from build123d import *

# Parameters (mm, degrees)
SKETCH2_R           = 31
BOSS_EXTRUDE1_DEPTH = 3
SKETCH3_R           = 22.5
BOSS_EXTRUDE2_DEPTH = 12
SKETCH4_R           = 17.5
CUT_EXTRUDE1_DEPTH  = 9
SKETCH6_R           = 2.75
CUT_EXTRUDE2_DEPTH  = 12


with BuildPart() as part:
    # Sketch2 → Boss-Extrude1 (new body)
    with BuildSketch(Plane.XY.offset(-694.189912682)):
        with Locations((-50, 0)):
            Circle(SKETCH2_R)
    extrude(amount=BOSS_EXTRUDE1_DEPTH)

    # Sketch3 → Boss-Extrude2 (add)
    with BuildSketch(Plane(origin=(0, 0, -694.189912682), x_dir=(-1, 0, 0), z_dir=(0, 0, -1))):
        with Locations((50, 0)):
            Circle(SKETCH3_R)
    extrude(amount=BOSS_EXTRUDE2_DEPTH)

    # Sketch4 → Cut-Extrude1 (cut)
    with BuildSketch(Plane(origin=(0, 0, -706.189912682), x_dir=(-1, 0, 0), z_dir=(0, 0, -1))):
        with Locations((50, 0)):
            Circle(SKETCH4_R)
    extrude(amount=-CUT_EXTRUDE1_DEPTH, mode=Mode.SUBTRACT)

    # Sketch6 → Cut-Extrude2 (cut)
    with BuildSketch(Plane.XY.offset(-691.189912682)):
        with Locations((-50, 26)):
            Circle(SKETCH6_R)
        with Locations((-24, 0)):
            Circle(SKETCH6_R)
        with Locations((-50, -26)):
            Circle(SKETCH6_R)
        with Locations((-76, 0)):
            Circle(SKETCH6_R)
    extrude(amount=-CUT_EXTRUDE2_DEPTH, mode=Mode.SUBTRACT)


solid = part.part
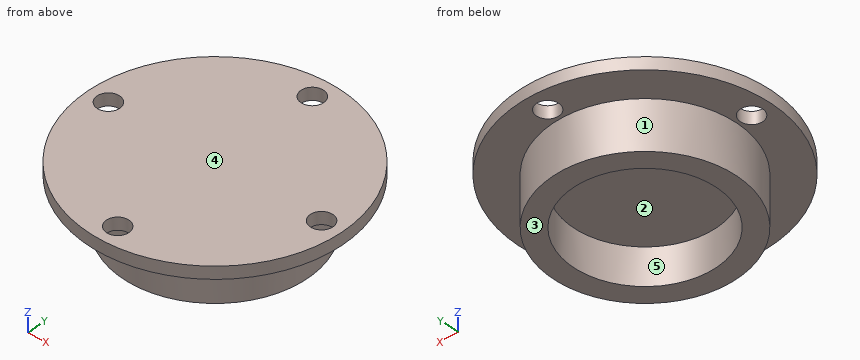
Work out the finished part from the listing and answer in its coordinate system (mm). Face numbers are marked on the shaded views. A direction names the side the tool comes from. Round coordinates to 2 decimals unless told otherwise and drop trailing zeros. Loops run counter-clockwise (first coordinate to the right, second up) from the corner with the lowest first, then second, coordinate; pieces in that order, holes last. Notation, with made-up numbers: (72.25, 72.25) - (94.25, 72.25) arc R18 cw to (94.25, 80.25) - close; hole circle Ø3 at (-24.5, 64). An arc over 180 degrees is marked (long way). Use one line per item in the form item = value. Start each with the question number.
(1) Find section A-A on x = -50. Determine the outline of the cut face in (y, z).
(2) Flat-ended cylindrical pins translate along their axes: P1, Ø4, axis at y = 8, z = -697, coming from the +X side; P2, Ø9, axis at x = -76, y = 0, coming from the -Z side; P3, Ø6, axis at x = -75, z = -695, coming from the +Y side; P4, Ø3, axis at y = 3.5, z = -697.5, coming from the +X side. Find the tip coordinate at first contact, or state that the pin passes through.
(3) Find section D-D on z = -699.25. Determine the outline of the cut face in (x, y).
(4) Consider line 1 (Y direction, x = -50, z = -693); line 2 (Z direction, x = -39.5, y = -27); line 3 (X direction, y = 10.5, z = -699.5). Determine where each line is inside the solid, lowest interval first.
(5) Determine the mould class of the marked faces 1, 2 and 3 for opening direction Y: +Y half, -Y half, draft (parallel to the pull), parting line (faces both ways), or undercut.
(6) Find section B-B on y = -26. Determine the outline of the cut face in (x, z), and give its area (3 significant figures).
(7) Which of the six approach directions +Z, -Z, +X, -X, +Y, -Y give full straight-line access (tool end or side, diameter ignored) to the marked faces 4 and 5?
(8) Find section C-C on x = -22.5. Determine the outline of the cut face in (y, z).
Answer list:
q1.outline = (-31, -694.19) - (-28.75, -694.19) - (-28.75, -691.19) - (-31, -691.19) - close; (-23.25, -694.19) - (-22.5, -694.19) - (-22.5, -706.19) - (-17.5, -706.19) - (-17.5, -697.19) - (17.5, -697.19) - (17.5, -706.19) - (22.5, -706.19) - (22.5, -694.19) - (23.25, -694.19) - (23.25, -691.19) - (-23.25, -691.19) - close; (28.75, -694.19) - (31, -694.19) - (31, -691.19) - (28.75, -691.19) - close
q2.P1 = -28.31
q2.P2 = -706.19
q2.P3 = 21.73
q2.P4 = -27.59
q3.outline = circle Ø45 at (-50, 0); hole circle Ø35 at (-50, 0)
q4.line_1 = -31 to -28.75, -23.25 to 23.25, 28.75 to 31
q4.line_2 = -694.19 to -691.19
q4.line_3 = -69.9 to -64, -36 to -30.1
q5.face_1 = parting line
q5.face_2 = undercut
q5.face_3 = draft
q6.outline = (-66.88, -694.19) - (-52.75, -694.19) - (-52.75, -691.19) - (-66.88, -691.19) - close; (-47.25, -694.19) - (-33.12, -694.19) - (-33.12, -691.19) - (-47.25, -691.19) - close
q6.area = 84.8 mm^2
q7.face_4 = +Z, +X, -X, +Y, -Y
q7.face_5 = -Z
q8.outline = (-14.31, -694.19) - (-2.3, -694.19) - (-2.3, -691.19) - (-14.31, -691.19) - close; (2.3, -694.19) - (14.31, -694.19) - (14.31, -691.19) - (2.3, -691.19) - close
